For this review, take the finished solid that the model builds, in its own axes (mm). Face numbers are marked on the shaded views. Coordinates: 2 decimals unless noted, no trailing zeros. Write each loop counter-clockwise with the first axis right and the second up, starting at its lowest first coordinate (ties: lowest second). Pieces come first, ordered by that corner, then holes.
1) Insertion check: P1, Ø4, axis at x = 1, y = 2.5, coming from the -Z side; P2, Ø1, axis at y = -1.5, z = 1.5, coming from the +X side. Each pin has a flat end and moves straight along its axis. Give the tip position at first contact, or say it passes through.
2) We need section D-D on x = -5.5. Write out the cut boundary in (y, z).
3) We need section B-B on y = -0.5. Write out the cut boundary in (x, z), then the cut area to 3 significant figures.
4) Mouldability with a two-part tool opening along X and no side actions: class the marked faces 1, 2 and 3 as pulls with the +X half, pulls with the -X half, needs draft (parallel to the pull), parting line crosses it, or undercut.
5) We need section C-C on z = 0.85. Write out the cut boundary in (x, y), then the cut area to 3 significant figures.
6) To check wall thickness, follow line 1 along Y through (x, z) = (0, 1); line 2 along Y through (x, z) = (-1.75, 0.35); line 3 along X through (y, z) = (-5, 1.25). State the ranges of each line that lie inside material, in increasing order.
7) We need section A-A on x = 0. Write out the cut boundary in (y, z).
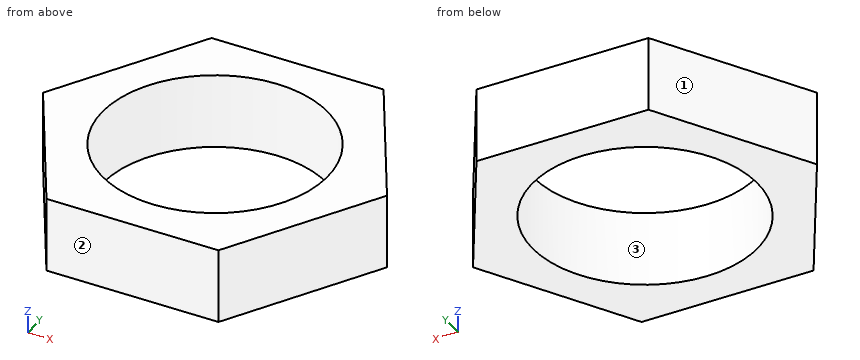
from build123d import *

# Parameters (mm, degrees)
BOSS_EXTRUDE1_DEPTH        = 3
M10X1_0_TAPPED_HOLE1_D     = 9
M10X1_0_TAPPED_HOLE1_DEPTH = 23
M10X1_0_TAPPED_HOLE1_TIP   = 2.703872786


with BuildPart() as part:
    # Sketch1 → Boss-Extrude1 (new body)
    with BuildSketch(Plane.XY):
        Polygon((6.92820323, 0), (3.464101615, 6), (-3.464101615, 6), (-6.92820323, 0), (-3.464101615, -6), (3.464101615, -6), align=None)
    extrude(amount=BOSS_EXTRUDE1_DEPTH)

    # M10x1.0 Tapped Hole1
    with Locations(Plane.XY.offset(3)):
        with Locations((0, 0)):
            Hole(M10X1_0_TAPPED_HOLE1_D / 2, depth=M10X1_0_TAPPED_HOLE1_DEPTH)
            with Locations((0, 0, -(M10X1_0_TAPPED_HOLE1_DEPTH + M10X1_0_TAPPED_HOLE1_TIP / 2))):  # 118° drill point
                Cone(0, M10X1_0_TAPPED_HOLE1_D / 2, M10X1_0_TAPPED_HOLE1_TIP, mode=Mode.SUBTRACT)


solid = part.part
Result:
1. P1: stops at z = 0
1. P2: stops at x = 6.35
2. outline: (-2.47, 0) - (2.47, 0) - (2.47, 3) - (-2.47, 3) - close
3. outline: (-6.64, 0) - (-4.47, 0) - (-4.47, 3) - (-6.64, 3) - close; (4.47, 0) - (6.64, 0) - (6.64, 3) - (4.47, 3) - close
3. area: 13.0 mm2
4. face 1: pulls with the -X half
4. face 2: needs draft
4. face 3: undercut
5. outline: (-6.93, 0) - (-3.46, -6) - (3.46, -6) - (6.93, 0) - (3.46, 6) - (-3.46, 6) - close; hole circle Ø9 at (0, 0)
5. area: 61.1 mm2
6. line 1: y = -6 to -4.5, 4.5 to 6
6. line 2: y = -6 to -4.15, 4.15 to 6
6. line 3: x = -4.04 to 4.04
7. outline: (-6, 0) - (-4.5, 0) - (-4.5, 3) - (-6, 3) - close; (4.5, 0) - (6, 0) - (6, 3) - (4.5, 3) - close
